Geometry: final body of the model. Coordinates: model frame, mm. Face numbers are marked on the shaded views. A direction names the side the tool comes from. Coordinates: 2 decimals unless noted, no trailing zeros. Loops run counter-clockwise (first coordinate to the right, second up) from the corner with the lowest first, then second, coordinate; pieces in that order, holes last. Notation, with made-up numbers: (-19, 15) - (-7, 15) arc R33 ccw to (-7, 50) - close; hole circle Ø2 at (53, 26.5). An arc over 180 degrees is marked (long way). Put each result on its own line as item: value. Start each with the question number.
1) Section B-B on z = 2. Output: boundary loops of the cut face in (x, y), and give its area (3 significant figures).
2) Contact query for flat-ended pins moving along their axis: pin 1 Ø1.2 at (x, z) = (0, 2) entering from +Y (3 decimals); pin 2 Ø2 at (x, z) = (-8.5, 1.5) entering from -Y; pin 3 Ø1.6 at (x, y) = (4, -2.5) entering from +Z; pin 4 Ø1.5 at (x, z) = (5.5, 3) entering from +Y. Output: stop coordinate, or through.
3) Material intervals for line 1 along X through (y, z) = (-0.3, 2); line 2 along X through (y, z) = (-0.25, 1.6); line 3 along Y through (x, z) = (-3.5, 1.3), sorted ascending. Write a range as from..to.
4) Reachability of the marked faces 1, 2 and 3 from +Z, -Z, +X, -X, +Y, -Y: full face, straight path, thin tool, end or side. Return the list, or none.
5) Section A-A on x = -15. Output: boundary loops of the cut face in (y, z).
6) Section D-D on x = -2. Output: boundary loops of the cut face in (y, z).
7) Section C-C on y = 1. Output: boundary loops of the cut face in (x, z).
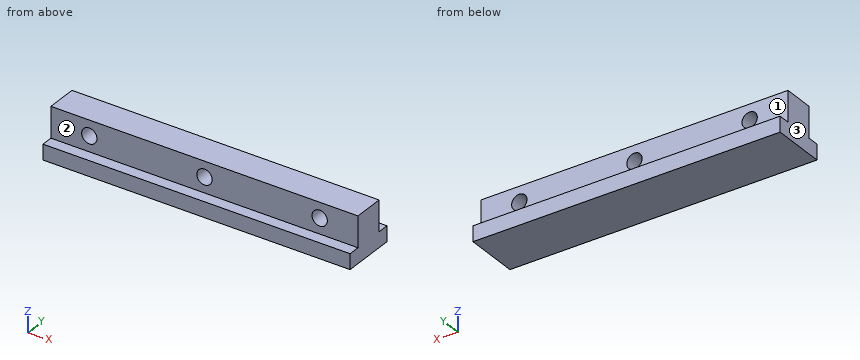
```python
from build123d import *

# Parameters (mm, degrees)
SKETCH_1_W          = 40
SKETCH_1_H          = 4
EXTRUDE_1_DEPTH     = 4
SKETCH_2_W          = 2
SKETCH_2_H          = 7
EXTRUDE_2_DEPTH     = 40
SKETCH_3_R          = 1
CUT_EXTRUDE_1_DEPTH = 22.124630174


with BuildPart() as part:
    # 草图1 → 凸台-拉伸1 (new body)
    with BuildSketch(Plane.XY):
        Rectangle(SKETCH_1_W, SKETCH_1_H)
    extrude(amount=EXTRUDE_1_DEPTH)

    # 草图2 → 凸台-拉伸2 (add)
    with BuildSketch(Plane(origin=(20, 0, 0), x_dir=(0, 0, -1), z_dir=(1, 0, 0))):
        with Locations((1, 0)):
            Rectangle(SKETCH_2_W, SKETCH_2_H)
    extrude(amount=-EXTRUDE_2_DEPTH)

    # 草图3 → 切除-拉伸1 (cut, through all)
    with BuildSketch(Plane(origin=(0, 2, 0), x_dir=(1, 0, 0), z_dir=(0, 1, 0))):
        with Locations(Location((-15, -2, 0), (0, 0, 270))):
            Circle(SKETCH_3_R)
        with Locations(Location((0, -2, 0), (0, 0, 270))):
            Circle(SKETCH_3_R)
        with Locations(Location((15, -2, 0), (0, 0, 270))):
            Circle(SKETCH_3_R)
    extrude(amount=-CUT_EXTRUDE_1_DEPTH, mode=Mode.SUBTRACT)


solid = part.part
```
Answer block:
1. outline: (-20, -2) - (-16, -2) - (-16, 2) - (-20, 2) - close; (-14, -2) - (-1, -2) - (-1, 2) - (-14, 2) - close; (1, -2) - (14, -2) - (14, 2) - (1, 2) - close; (16, -2) - (20, -2) - (20, 2) - (16, 2) - close
1. area: 136 mm²
2. pin 1: passes through
2. pin 2: stops at y = -2
2. pin 3: stops at z = 4
2. pin 4: stops at y = 2
3. line 1: x = -20..-16, -14..-1, 1..14, 16..20
3. line 2: x = -20..-15.92, -14.08..-0.92, 0.92..14.08, 15.92..20
3. line 3: y = -2..2
4. face 1: +Z, +X, -X, +Y
4. face 2: +Z, +X, -X, -Y
4. face 3: +Z, -Z, -X, +Y, -Y
5. outline: (-3.5, -2) - (3.5, -2) - (3.5, 0) - (2, 0) - (2, 1) - (-2, 1) - (-2, 0) - (-3.5, 0) - close; (-2, 3) - (2, 3) - (2, 4) - (-2, 4) - close
6. outline: (-3.5, -2) - (3.5, -2) - (3.5, 0) - (2, 0) - (2, 4) - (-2, 4) - (-2, 0) - (-3.5, 0) - close
7. outline: (-20, -2) - (20, -2) - (20, 4) - (-20, 4) - close; hole circle Ø2 at (-15, 2); hole circle Ø2 at (0, 2); hole circle Ø2 at (15, 2)
